```python
from build123d import *
from OCP.BRepFilletAPI import BRepFilletAPI_MakeChamfer

# Parameters (mm, degrees)
SKETCH1_R           = 18
BOSS_EXTRUDE1_DEPTH = 4
SKETCH2_R           = 8.5
BOSS_EXTRUDE2_DEPTH = 27
BOSS_EXTRUDE3_START = 27
SKETCH3_R           = 8
BOSS_EXTRUDE3_DEPTH = 20
CHAMFER1_SIZE       = 0.5
CHAMFER1_SIZE2      = 0.288675135
SKETCH4_R           = 2.75
CUT_EXTRUDE1_DEPTH  = 20


with BuildPart() as part:
    # Sketch1 → Boss-Extrude1 (new body)
    with BuildSketch(Plane.XY):
        Circle(SKETCH1_R)
    extrude(amount=BOSS_EXTRUDE1_DEPTH)

    # Sketch2 → Boss-Extrude2 (add)
    with BuildSketch(Plane.XY.offset(4)):
        Circle(SKETCH2_R)
    extrude(amount=BOSS_EXTRUDE2_DEPTH)

    # Sketch3 → Boss-Extrude3 (add)
    with BuildSketch(Plane.XY.offset(4).offset(BOSS_EXTRUDE3_START)):
        Circle(SKETCH3_R)
    extrude(amount=BOSS_EXTRUDE3_DEPTH)

    # Chamfer1: one chamfer whose edges measure the first distance from different faces: ONE call of the kernel's chamfer builder (chamfer() names one face for all edges)
    chamfer1_edges_1 = [part.edges().sort_by_distance(p)[0] for p in [
        (-8, 0, 51),
    ]]
    chamfer1_side_1 = [part.faces().sort_by_distance(p)[0] for p in [
        (-8, 0, 41),
    ]]
    chamfer1_edges_2 = [part.edges().sort_by_distance(p)[0] for p in [
        (-18, 0, 0),
    ]]
    chamfer1_side_2 = [part.faces().sort_by_distance(p)[0] for p in [
        (0, 0, 0),
    ]]
    chamfer1 = BRepFilletAPI_MakeChamfer(part.part.solid().wrapped)
    for e in chamfer1_edges_1:
        chamfer1.Add(CHAMFER1_SIZE, CHAMFER1_SIZE2, e.wrapped, chamfer1_side_1[0].wrapped)  # the first distance lies on this face
    for e in chamfer1_edges_2:
        chamfer1.Add(CHAMFER1_SIZE, CHAMFER1_SIZE2, e.wrapped, chamfer1_side_2[0].wrapped)  # the first distance lies on this face
    add(Compound.cast(chamfer1.Shape()), mode=Mode.REPLACE)

    # Sketch4 → Cut-Extrude1 (cut)
    with BuildSketch(Plane(origin=(0, 0, 0), x_dir=(-1, 0, 0), z_dir=(0, 0, -1))):
        with Locations((0, 12.5)):
            Circle(SKETCH4_R)
        with Locations((0, -12.5)):
            Circle(SKETCH4_R)
    extrude(amount=-CUT_EXTRUDE1_DEPTH, mode=Mode.SUBTRACT)


solid = part.part
```
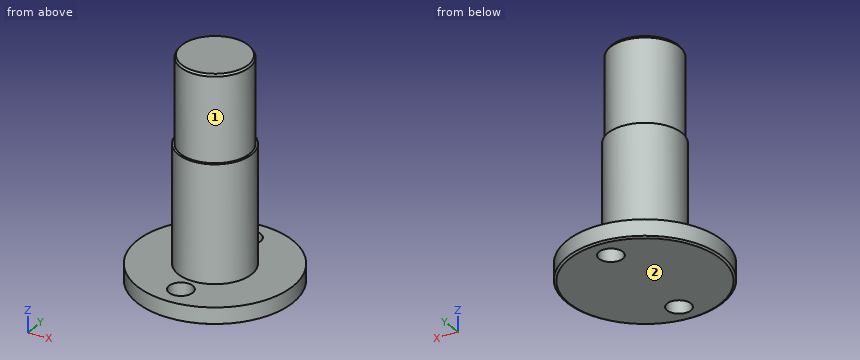
Source: CAD feature listing. Evaluate the final solid. Frame: model axes, mm. Face numbers are marked on the shaded views. A direction names the side the tool comes from. Coordinates: 2 decimals unless noted, no trailing zeros. Order: outer loops, then holes, each group sorted by start corner. A loop starts at its lowest first (then second) coordinate and runs counter-clockwise, first axis right, second up. Notation, with made-up numbers: (56.5, 43.25) - (84.5, 43.25) arc R23 ccw to (84.5, 64.25) - close; hole circle Ø3 at (0, -28). An arc over 180 degrees is marked (long way). One line per item, written item: value.
1) Cut plane A-A on x = 0. Output: boundary loops of the cut face in (y, z).
Computed values:
outline: (-18, 0.29) - (-17.5, 0) - (-15.25, 0) - (-15.25, 4) - (-18, 4) - close; (-9.75, 0) - (9.75, 0) - (9.75, 4) - (8.5, 4) - (8.5, 31) - (8, 31) - (8, 50.5) - (7.71, 51) - (-7.71, 51) - (-8, 50.5) - (-8, 31) - (-8.5, 31) - (-8.5, 4) - (-9.75, 4) - close; (15.25, 0) - (17.5, 0) - (18, 0.29) - (18, 4) - (15.25, 4) - close
2) Cut plane B-B on y = 0. Output: boundary loops of the cut face in (x, z).
Computed values:
outline: (-18, 0.29) - (-17.5, 0) - (17.5, 0) - (18, 0.29) - (18, 4) - (8.5, 4) - (8.5, 31) - (8, 31) - (8, 50.5) - (7.71, 51) - (-7.71, 51) - (-8, 50.5) - (-8, 31) - (-8.5, 31) - (-8.5, 4) - (-18, 4) - close
3) Ray query, line 1 (Y direction, x = 0, z = 2.6); line 2 (Z direction, x = 11.5, y = -2); line 3 (X direction, y = -12, z = 2). Return the intervals inside material, ascending. Write a range as [from, to].
Computed values:
line 1: y = [-18, -15.25], [-9.75, 9.75], [15.25, 18]
line 2: z = [0, 4]
line 3: x = [-13.42, -2.7], [2.7, 13.42]
4) Cut plane D-D on z = 11.5. Output: boundary loops of the cut face in (x, y), plus the area to 3 significant figures.
Computed values:
outline: circle Ø17 at (0, 0)
area: 227 mm^2
5) Reachability of the marked faces 1 and 2 from +Z, -Z, +X, -X, +Y, -Y: full face, straight path, thin tool, end or side. Return the list, or none.
Computed values:
face 1: +Z
face 2: -Z, +X, -X, +Y, -Y
6) Cut plane C-C on z = 32. Output: boundary loops of the cut face in (x, y), plus the area to 3 significant figures.
Computed values:
outline: circle Ø16 at (0, 0)
area: 201 mm^2
7) Contact query for flat-ended pins moving along their axis: pin 1 (1.5 mm diameter, centred on y = 7, z = 43, fed in from -X); pin 2 (6 mm diameter, centred on y = -5, z = 28, fed in from -X); pin 3 (2 mm diameter, centred on y = 7.5, z = 19, fed in from -X); pin 4 (5 mm diameter, centred on x = 0, y = -12.5, fed in from -Z). Output: stop coordinate, or through.
Computed values:
pin 1: stops at x = -4.99
pin 2: stops at x = -8.26
pin 3: stops at x = -5.48
pin 4: passes through
